```python
from build123d import *

# Parameters (mm, degrees)
SHELL1_T           = -2
SKETCH2_R          = 229
CUT_EXTRUDE1_DEPTH = 101
CUT_EXTRUDE2_DEPTH = 268
CIRPATTERN1_COUNT  = 6


with BuildPart() as part:
    # Sketch1 → Revolve1 (revolve)
    with BuildSketch(Plane.XY):
        Polygon((0, 0), (0, 790), (230, 790), (230, 650), (552, 650), (552, 318), (502, 318), (502, 0), align=None)
    revolve(axis=Axis((0, 0, 0), (0, 1, 0)))

    # Shell1
    shell1_openings = [part.faces().sort_by_distance(p)[0] for p in [
        (0, 0, 0),
    ]]
    offset(amount=SHELL1_T, openings=shell1_openings, kind=Kind.INTERSECTION)

    # Sketch2 → Cut-Extrude1 (cut)
    with BuildSketch(Plane(origin=(0, 790, 0), x_dir=(1, 0, 0), z_dir=(0, 1, 0))):
        with Locations(Location((0, 0, 0), (0, 0, 180))):
            Circle(SKETCH2_R)
    extrude(amount=-CUT_EXTRUDE1_DEPTH, mode=Mode.SUBTRACT)

    # Sketch3 → Cut-Extrude2 (cut)
    with BuildSketch(Plane(origin=(0, 0, 0), x_dir=(1, 0, 0), z_dir=(0, 1, 0))):
        Polygon((0, 0), (635.384163394, 0), (612.361562027, -189.37712274), align=None)
    cut_extrude2 = extrude(amount=CUT_EXTRUDE2_DEPTH, mode=Mode.SUBTRACT)

    # CirPattern1: Cut-Extrude2 ×6 about axis
    cirpattern1_axis = Axis((0, 0, 0), (0, 1, 0))
    for i in range(1, CIRPATTERN1_COUNT):
        add(cut_extrude2.rotate(cirpattern1_axis, i * 360 / CIRPATTERN1_COUNT), mode=Mode.SUBTRACT)


solid = part.part
```
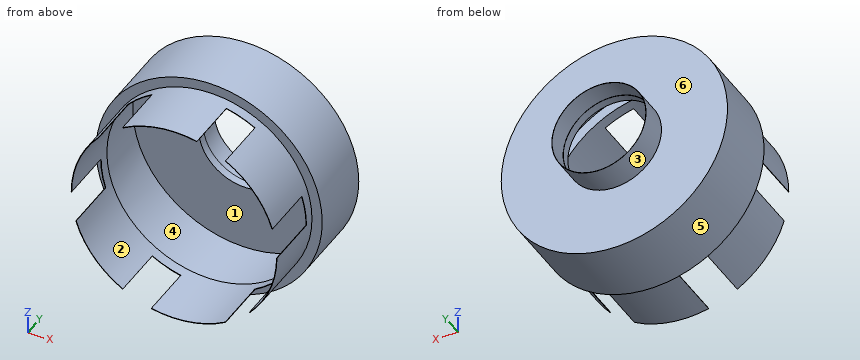
Work out the finished part from the listing and answer in its coordinate system (mm). Face numbers are marked on the shaded views. A direction names the side the tool comes from. Round coordinates to 2 decimals unless told otherwise and drop trailing zeros. Loops run counter-clockwise (first coordinate to the right, second up) from the corner with the lowest first, then second, coordinate; pieces in that order, holes last.
(1) The mould has two halves that part along Z. Classify the marked faces 4, 5 and 6: pulls with the +Z half, pulls with the -Z half, needs draft (parallel to the pull), parting line crosses it, or undercut.
Computed values:
face 4: undercut
face 5: parting line crosses it
face 6: needs draft
(2) The part is cut by section C-C, the plane z = -17.5. Give the vertices of the cut face in (x, y).
Computed values:
outline: (-551.72, 318) - (-501.69, 318) - (-501.69, 268) - (-499.69, 268) - (-499.69, 320) - (-549.72, 320) - (-549.72, 648) - (-227.33, 648) - (-227.33, 689) - (-228.33, 689) - (-228.33, 790) - (-229.33, 790) - (-229.33, 650) - (-551.72, 650) - close; (227.33, 648) - (549.72, 648) - (549.72, 320) - (499.69, 320) - (499.69, 0) - (501.69, 0) - (501.69, 318) - (551.72, 318) - (551.72, 650) - (229.33, 650) - (229.33, 790) - (228.33, 790) - (228.33, 689) - (227.33, 689) - close
(3) Find the intervals of material crossed by L1, parallel to Z at x = -8, y = 516; L2, parallel to Y at x = -480.5, z = 260; L3, parallel to Z at x = 0, y = 730, in increasing order.
Computed values:
L1: z = -551.94 to -549.94, 549.94 to 551.94
L2: y = 318 to 320, 648 to 650
L3: z = -230 to -229, 229 to 230
(4) Each of these flat-tipped pins is pushed along its axis until it touches: P1, Ø1.6, axis at x = -500.5, y = 92, coming from the -Z side; P2, Ø5, axis at y = 686, z = 112, coming from the -X side; P3, Ø1, axis at x = 348.5, y = 511.5, coming from the +Z side. Where does it stop, or does it pass through?
Computed values:
P1: stops at z = 0
P2: stops at x = -202.26
P3: stops at z = 428.49
(5) The part is cut by section D-D, the plane y = 464. Give the vertices of the cut face in (x, z).
Computed values:
outline: circle Ø1104 at (0, 0); hole circle Ø1100 at (0, 0)
(6) The part is cut by section A-A, the plane x = 0. Give the vertices of the cut face in (y, z).
Computed values:
outline: (0, -502) - (318, -502) - (318, -552) - (650, -552) - (650, -230) - (790, -230) - (790, -229) - (689, -229) - (689, -228) - (648, -228) - (648, -550) - (320, -550) - (320, -500) - (0, -500) - close; (0, 500) - (320, 500) - (320, 550) - (648, 550) - (648, 228) - (689, 228) - (689, 229) - (790, 229) - (790, 230) - (650, 230) - (650, 552) - (318, 552) - (318, 502) - (0, 502) - close
(7) For the marked faces 1, 2 and 3, determine the directions among +Z, -Z, +X, -X, +Y, -Y from which every point of the face is accessible in a straight line to the end or side of a thin tool.
Computed values:
face 1: none
face 2: -Y
face 3: +Y
(8) The part is cut by section B-B, the plane y = 157. Give the vertices of the cut face in (x, z), and give its area (3 significant figures).
Computed values:
outline: (-502, 0) - (-500, 0) arc R500 cw to (-366.77, 339.82) - (-368.24, 341.18) arc R502 ccw to start; (-479.59, -148.32) arc R502 ccw to (-251, -434.74) - (-250, -433.01) arc R500 cw to (-477.68, -147.73) - close; (-251, 434.74) - (-250, 433.01) arc R500 cw to (110.91, 487.54) - (111.35, 489.5) arc R502 ccw to start; (-111.35, -489.5) arc R502 ccw to (251, -434.74) - (250, -433.01) arc R500 cw to (-110.91, -487.54) - close; (250, 433.01) arc R500 cw to (477.68, 147.73) - (479.59, 148.32) arc R502 ccw to (251, 434.74) - close; (366.77, -339.82) - (368.24, -341.18) arc R502 ccw to (502, 0) - (500, 0) arc R500 cw to start
area: 4,490 mm2
